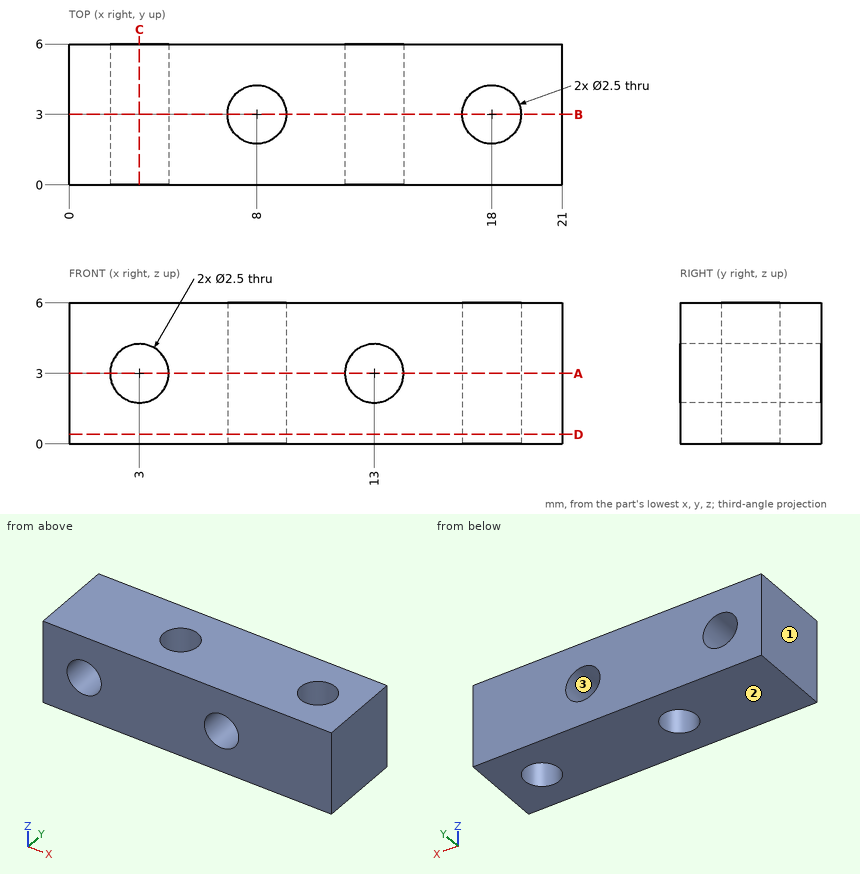
The drawing under review shows one solid part. Ordinate dimensions are in mm from its lowest x, y, z. Give positions to 0.01 mm unless a question says otherwise; leave off trailing zeros. Loops run counter-clockwise (first coordinate to the right, second up) from the corner with the lowest first, then second, coordinate; pieces in that order, holes last. Notation, with made-up numbers: M -18,70 L 14,70 A21 cw 14,76 Z; hole C 51,61 d8. An arc over 180 degrees is marked long. Return JSON: item names as keys, results as strings. Group by question number.
Item 1: Mouldability with a two-part tool opening along X and no side actions: class the marked faces 1, 2 and 3 as released by +X, released by -X, zero draft, split by the parting line, or undercut.
Item 2: We need section A-A (z = 3). Give the boundary of the cut face in (x, y), and give its area (3 significant figures).
Item 3: We need section D-D (z = 0.4). Give the boundary of the cut face in (x, y).
Item 4: For probe 1 along Z at (x, y) = (3, 4.1); probe 2 along X at (y, z) = (4.3, 3.8); probe 3 along X at (y, z) = (3.65, 4.35), list the stretches that pass through material, from the lowest coordinate up.
Item 5: Insertion check: pin 1 Ø2 at (x, z) = (3, 3) entering from +Y. The pin has a flat end and moves straight along its axis. Give the tip position at first contact, or say it passes through.
Item 6: We need section B-B (y = 3). Give the boundary of the cut face in (x, z).
Item 7: We need section C-C (x = 3). Give the boundary of the cut face in (y, z), and give its area (3 significant figures).
Output:
{
 "1": {"face 1": "released by -X", "face 2": "zero draft", "face 3": "undercut"},
 "2": {"outline": "M 0,0 L 1.75,0 L 1.75,6 L 0,6 Z; M 4.25,0 L 11.75,0 L 11.75,6 L 4.25,6 Z; M 14.25,0 L 21,0 L 21,6 L 14.25,6 Z; hole C 8,3 d2.5; hole C 18,3 d2.5", "area": "86.2 mm^2"},
 "3": {"outline": "M 0,0 L 21,0 L 21,6 L 0,6 Z; hole C 8,3 d2.5; hole C 18,3 d2.5"},
 "4": {"probe 1": "z = 0 to 1.75, 4.25 to 6", "probe 2": "x = 0 to 2.04, 3.96 to 12.04, 13.96 to 21", "probe 3": "x = 0 to 6.93, 9.07 to 16.93, 19.07 to 21"},
 "5": {"pin 1": "passes through"},
 "6": {"outline": "M 0,0 L 6.75,0 L 6.75,6 L 0,6 Z; M 9.25,0 L 16.75,0 L 16.75,6 L 9.25,6 Z; M 19.25,0 L 21,0 L 21,6 L 19.25,6 Z; hole C 3,3 d2.5; hole C 13,3 d2.5"},
 "7": {"outline": "M 0,0 L 6,0 L 6,1.75 L 0,1.75 Z; M 0,4.25 L 6,4.25 L 6,6 L 0,6 Z", "area": "21.0 mm^2"}
}
